Here's how the part is built. I have some questions about the finished solid (model axes, mm). Coordinates: 2 decimals unless noted, no trailing zeros. Write each loop counter-clockwise with the first axis right and the second up, starting at its lowest first coordinate (ties: lowest second). Pieces come first, ordered by that corner, then holes. Notation, with made-up numbers: M 21,3 L 25,3 A10 ccw 25,12 Z; hole C -30.5,-30 d7. An arc over 180 degrees is marked long. Use a Markdown table: item, result.
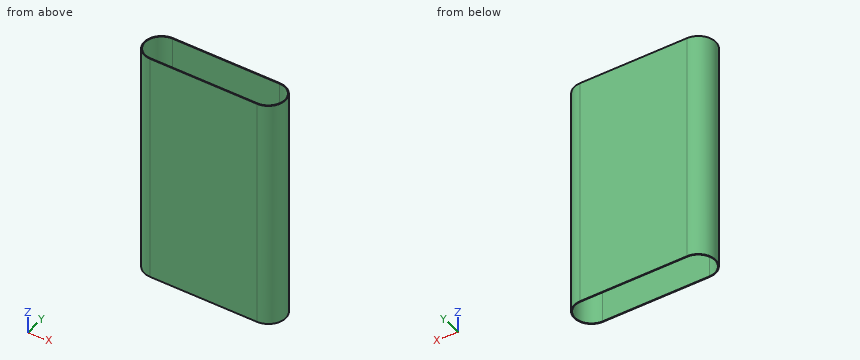
```python
from build123d import *

# Parameters (mm, degrees)
EXTRUDE_1_DEPTH = 850


with BuildPart() as part:
    # 草图1 → 凸台-拉伸1 (new body)
    with BuildSketch(Plane(origin=(0, 0, 425), x_dir=(-1, 0, 0), z_dir=(0, 0, -1))):
        with BuildLine():
            Line((-601.038579668, 1587.00944222), (-201.099501606, 1593.990404795))
            ThreePointArc((-201.099501606, 1593.990404795), (-137.009595205, 1532.099501606), (-198.900498394, 1468.009595205))
            Line((-198.900498394, 1468.009595205), (-598.839576457, 1461.02863263))
            ThreePointArc((-598.839576457, 1461.02863263), (-662.929482857, 1522.91953582), (-601.038579668, 1587.00944222))
        make_face()
        with BuildLine():
            Line((-600.986222449, 1584.009899134), (-201.047144386, 1590.990861709))
            ThreePointArc((-201.047144386, 1590.990861709), (-140.009138291, 1532.047144386), (-198.952855614, 1471.009138291))
            Line((-198.952855614, 1471.009138291), (-598.891933676, 1464.028175716))
            ThreePointArc((-598.891933676, 1464.028175716), (-659.929939772, 1522.971893039), (-600.986222449, 1584.009899134))
        make_face(mode=Mode.SUBTRACT)
    extrude(amount=EXTRUDE_1_DEPTH)


solid = part.part
```
1. Suppose I cut it at A-A on z = -365. Write out the boundary of the cut face in (x, y), and give its area (3 significant figures).
Answers follow:
| item | result |
|---|---|
| outline | M 198.9,1468.01 L 598.84,1461.03 A63 ccw 601.04,1587.01 L 201.1,1593.99 A63 ccw Z; hole M 198.95,1471.01 L 598.89,1464.03 A60 ccw 600.99,1584.01 L 201.05,1590.99 A60 ccw Z |
| area | 3,560 mm2 |
2. Suppose I cut it at C-C on x = 214.5. Write out the boundary of the cut face in (y, z), and give its area (3 significant figures).
Answers follow:
| item | result |
|---|---|
| outline | M 1467.74,-425 L 1470.74,-425 L 1470.74,425 L 1467.74,425 Z; M 1590.76,-425 L 1593.76,-425 L 1593.76,425 L 1590.76,425 Z |
| area | 5,100 mm2 |
3. Suppose I cut it at B-B on y = 1571. Write out the boundary of the cut face in (x, z).
Answers follow:
| item | result |
|---|---|
| outline | M 151.33,-425 L 155.28,-425 L 155.28,425 L 151.33,425 Z; M 637.26,-425 L 641.91,-425 L 641.91,425 L 637.26,425 Z |
4. I need wall thicknesses on probe 1 along Y at (x, z) = (209, -15.5); probe 2 along Y at (x, z) = (205, 77); probe 3 along X at (y, z) = (1562, 181). Which ranges of each line are inside material? Lowest first, please.
Answers follow:
| item | result |
|---|---|
| probe 1 | y = 1467.83 to 1470.83, 1590.85 to 1593.85 |
| probe 2 | y = 1467.9 to 1470.9, 1590.92 to 1593.92 |
| probe 3 | x = 145.15 to 148.63, 646.39 to 650.2 |
5. Will these pins go through, and if not, where does the flat tip stop? pin 1 Ø6 at (y, z) = (1533, -300) entering from -X; pin 2 Ø6 at (y, z) = (1493, 318.5) entering from +X; pin 3 Ø8 at (y, z) = (1497, 180) entering from +X; pin 4 Ø6 at (x, z) = (259, 241) entering from -Y.
Answers follow:
| item | result |
|---|---|
| pin 1 | stops at x = 137 |
| pin 2 | stops at x = 656.37 |
| pin 3 | stops at x = 658.58 |
| pin 4 | stops at y = 1466.91 |
